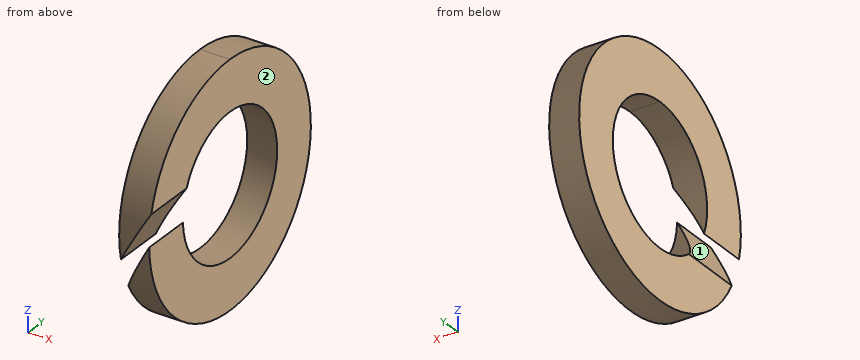
from build123d import *

# Parameters (mm, degrees)
SKETCH1_W          = 3
SKETCH1_H          = 5
CUT_EXTRUDE1_REACH = 24.972


with BuildPart() as part:
    # Sketch1 → Revolve1 (revolve)
    with BuildSketch(Plane.XY, mode=Mode.PRIVATE) as revolve1_sk:
        with Locations((13.982621868, 9.5)):
            Rectangle(SKETCH1_W, SKETCH1_H)
    revolve(revolve1_sk.sketch.rotate(Axis((0, 0, 0), (1, 0, 0)), 90), axis=Axis((0, 0, 0), (1, 0, 0)))

    # Sketch3 → Cut-Extrude1 (cut, up to next)
    with BuildSketch(Plane(origin=(0, 0, 0), x_dir=(1, 0, 0), z_dir=(0, 1, 0)), mode=Mode.PRIVATE) as cut_extrude1_sk1:
        Polygon((7.694741439, 13.902815003), (23.953594269, -14.55017745), (22.65325389, -15.293229095), (5.96980012, 13.902815003), align=None)
    cut_extrude1_tool1 = extrude(cut_extrude1_sk1.sketch, amount=-CUT_EXTRUDE1_REACH, mode=Mode.PRIVATE) & part.part
    add(cut_extrude1_tool1.solids().sort_by_distance((15.064598, 0, 0.510242))[0], mode=Mode.SUBTRACT)


solid = part.part
For this review, take the finished solid that the model builds, in its own axes (mm). Face numbers are marked on the shaded views. Coordinates: 2 decimals unless noted, no trailing zeros. Loops run counter-clockwise (first coordinate to the right, second up) from the corner with the lowest first, then second, coordinate; pieces in that order, holes last. Notation, with made-up numbers: (89.5, 66.25) - (144.5, 66.25) arc R11 cw to (144.5, 86.25) - close; hole circle Ø7 at (-22.75, 30). An arc over 180 degrees is marked (long way). Return JSON: item names as keys, results as strings.
Item 1: Take a section at B-B (y = 2). Give the boundary of the cut face in (x, z).
Determined:
{"outline": "(12.48, -11.83) - (15.48, -11.83) - (15.48, -6.71) - (12.48, -6.71) - close; (12.48, 6.71) - (15.48, 6.71) - (15.48, 11.83) - (12.48, 11.83) - close"}
Item 2: Take a section at A-A (z = -4.5). Give the boundary of the cut face in (x, y), then the cut area to 3 significant figures.
Determined:
{"outline": "(12.48, 5.36) - (15.48, 5.36) - (15.48, 11.12) - (12.48, 11.12) - close; (13.07, -11.12) - (15.48, -11.12) - (15.48, -5.36) - (13.07, -5.36) - close", "area": "31.2 mm2"}
Item 3: Insertion check: pin 1 (1 mm diameter, centred on x = 14, z = 9, fed in from +Y); pin 2 (4 mm diameter, centred on y = -5, z = -5.5, fed in from -X). Each pin has a flat end and moves straight along its axis. Give the tip position at first contact, or say it passes through.
Determined:
{"pin 1": "stops at y = 8.47", "pin 2": "stops at x = 12.48"}
Item 4: Take a section at C-C (x = 14.65). Give the boundary of the cut face in (y, z), then the cut area to 3 significant figures.
Determined:
{"outline": "(-11.93, 1.29) - (-6.88, 1.29) arc R7 cw (long way) to (-6.78, -1.73) - (-11.87, -1.73) arc R12 ccw (long way) to start", "area": "283 mm2"}
Item 5: Mouldability with a two-part tool opening along Z and no side actions: class the marked faces 1 and 2 as pulls with the +Z half, pulls with the -Z half, needs draft (parallel to the pull), parting line crosses it, or undercut.
Determined:
{"face 1": "undercut", "face 2": "needs draft"}
Item 6: For line 1 (Y direction, x = 13.2, z = 0); line 2 (Z direction, x = 14.7, y = -9.75); line 3 (Y direction, x = 14.6, z = 0), list the stretches that pass through material, from the lowest coordinate up.
Determined:
{"line 1": "y = -12 to -7, 7 to 12", "line 2": "z = -7 to -1.64, 1.38 to 7", "line 3": "y = 7 to 12"}
Item 7: Take a section at D-D (z = -7.5). Give the boundary of the cut face in (x, y), then the cut area to 3 significant figures.
Determined:
{"outline": "(12.48, -9.37) - (15.48, -9.37) - (15.48, 9.37) - (12.48, 9.37) - close", "area": "56.2 mm2"}
